The model under review builds one solid part; all positions refer to its coordinate system, in mm. Face numbers are marked on the shaded views. A direction names the side the tool comes from. Coordinates: 2 decimals unless noted, no trailing zeros. Loops run counter-clockwise (first coordinate to the right, second up) from the corner with the lowest first, then second, coordinate; pieces in that order, holes last. Notation, with made-up numbers: (84, 39) - (99, 39) arc R15 cw to (99, 50) - close; hole circle Ø9 at (57.25, -39). An arc over 180 degrees is marked (long way). Answer in a Markdown table with one row per item. Add a question column.
(1) We need section C-C on z = 322.5. Write out the cut boundary in (x, y), plus the area to 3 significant figures.
(2) We need section D-D on x = 241.5. Write out the cut boundary in (y, z).
(3) Mouldability with a two-part tool opening along X and no side actions: class the marked faces 1, 2 and 3 as +X half, -X half, draft (parallel to the pull), parting line (faces both ways), or undercut.
(4) We need section B-B on y = 42. Write out the cut boundary in (x, z).
(5) We need section A-A on z = 81.5. Write out the cut boundary in (x, y), plus the area to 3 significant figures.
(6) For P1, Ø6, axis at y = -32.5, z = 304.5, coming from the -X side; P2, Ø13.5, axis at x = 303, z = 61.5, coming from the -Y side; P3, Ø1.6, axis at x = 279.5, y = 27.5, coming from the -Z side, all flat-tipped, find the tip position at first contact; note any pin that passes through.
(7) Machinability: for the marked faces 4 and 5, which of the approach directions +Z, -Z, +X, -X, +Y, -Y give a long, thin tool a straight path to every point of the face, cutting with its end or side? Answer none if there is none.
(8) For line 1 along Z through (x, y) = (313.5, 110.8); line 2 along Y through (x, z) = (188, 140.5); line 3 along X through (y, z) = (111.05, 110), list the stretches that pass through material, from the lowest coordinate up.
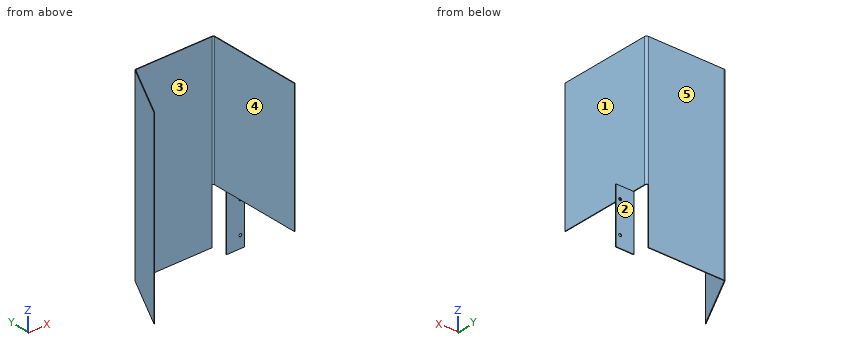
from build123d import *

# Parameters (mm, degrees)
BOSS_EXTRUDE1_DEPTH = 470
SKETCH2_W           = 259.384711363
SKETCH2_H           = 314.468537248
CUT_EXTRUDE3_DEPTH  = 1.5
SKETCH5_W           = 57.928223487
SKETCH5_H           = 140
CUT_EXTRUDE9_DEPTH  = 58.5
SKETCH7_W           = 48.5
SKETCH7_H           = 140
BOSS_EXTRUDE3_DEPTH = 1.5
MOVE_FACE1_BY       = 3.5
SKETCH9_R           = 3.5
CUT_EXTRUDE10_DEPTH = 1.5


with BuildPart() as part:
    # Sketch1 → Boss-Extrude1 (new body)
    with BuildSketch(Plane.XY):
        with BuildLine():
            Line((0, 0), (78.588235294, 147.352941176))
            ThreePointArc((78.588235294, 147.352941176), (80.427521223, 149.287464629), (83, 150))
            Line((83, 150), (275, 150))
            ThreePointArc((275, 150), (278.535533906, 148.535533906), (280, 145))
            Line((280, 145), (280, -90))
            Line((280, -90), (278.5, -90))
            Line((278.5, -90), (278.5, 145))
            ThreePointArc((278.5, 145), (277.474873734, 147.474873734), (275, 148.5))
            Line((275, 148.5), (83, 148.5))
            ThreePointArc((83, 148.5), (81.199264856, 148.00122524), (79.911764706, 146.647058824))
            Line((79.911764706, 146.647058824), (1.7, 0))
            Line((1.7, 0), (0, 0))
        make_face()
    extrude(amount=BOSS_EXTRUDE1_DEPTH)

    # Sketch2 → Cut-Extrude3 (cut)
    with BuildSketch(Plane.ZY.offset(-278.5)):
        with Locations((10.307644318, -12.234268624)):
            Rectangle(SKETCH2_W, SKETCH2_H)
    extrude(amount=-CUT_EXTRUDE3_DEPTH, mode=Mode.SUBTRACT)

    # Sketch5 → Cut-Extrude9 (cut)
    with BuildSketch(Plane(origin=(0, 150, 0), x_dir=(1, 0, 0), z_dir=(0, 1, 0))):
        with Locations((303.964111743, -70)):
            Rectangle(SKETCH5_W, SKETCH5_H)
    extrude(amount=-CUT_EXTRUDE9_DEPTH, mode=Mode.SUBTRACT)

    # Sketch7 → Boss-Extrude3 (add)
    with BuildSketch(Plane(origin=(0, 110, 0), x_dir=(1, 0, 0), z_dir=(0, 1, 0))):
        with Locations((299.25, -70)):
            Rectangle(SKETCH7_W, SKETCH7_H)
    extrude(amount=BOSS_EXTRUDE3_DEPTH)

    # Move Face1: a face moved inward by 3.5
    extrude(part.faces().sort_by_distance((275, 110.75, 70))[0], amount=MOVE_FACE1_BY, dir=(1, 0, 0), mode=Mode.SUBTRACT)

    # Sketch9 → Cut-Extrude10 (cut)
    with BuildSketch(Plane(origin=(0, 111.5, 0), x_dir=(1, 0, 0), z_dir=(0, 1, 0))):
        with Locations(Location((313.5, -30, 0), (0, 0, 270))):
            Circle(SKETCH9_R)
        with Locations(Location((313.5, -110, 0), (0, 0, 270))):
            Circle(SKETCH9_R)
    extrude(amount=-CUT_EXTRUDE10_DEPTH, mode=Mode.SUBTRACT)


solid = part.part
Outcome:
| question | item | result |
|---|---|---|
| 1 | outline | (0, 0) - (1.7, 0) - (79.91, 146.65) arc R3.5 cw to (83, 148.5) - (275, 148.5) arc R3.5 cw to (278.5, 145) - (278.5, -90) - (280, -90) - (280, 145) arc R5 ccw to (275, 150) - (83, 150) arc R5 ccw to (78.59, 147.35) - close |
| 1 | area | 907 mm² |
| 2 | outline | (148.5, 0) - (150, 0) - (150, 470) - (148.5, 470) - close |
| 3 | face 1 | +X half |
| 3 | face 2 | draft |
| 3 | face 3 | undercut |
| 4 | outline | (22.4, 0) - (24.1, 0) - (24.1, 470) - (22.4, 470) - close; (278.5, 140) - (280, 140) - (280, 470) - (278.5, 470) - close |
| 5 | outline | (0, 0) - (1.7, 0) - (79.91, 146.65) arc R3.5 cw to (83, 148.5) - (275, 148.5) - (275, 150) - (83, 150) arc R5 ccw to (78.59, 147.35) - close; (278.5, 110) - (323.5, 110) - (323.5, 111.5) - (278.5, 111.5) - close |
| 5 | area | 612 mm² |
| 6 | P1 | x = 278.5 |
| 6 | P2 | y = 110 |
| 6 | P3 | z = 140 |
| 7 | face 4 | +Z, -Z, -Y |
| 7 | face 5 | +Z, -Z, +X, -X, +Y |
| 8 | line 1 | 0 to 26.5, 33.5 to 106.5, 113.5 to 140 |
| 8 | line 2 | 148.5 to 150 |
| 8 | line 3 | 59.23 to 60.93, 278.5 to 310, 317 to 323.5 |
